```python
from build123d import *

# Parameters (mm, degrees)
SKETCH_1_W          = 200
SKETCH_1_H          = 30
EXTRUDE_1_DEPTH     = 12
SKETCH_2_W          = 12
SKETCH_2_H          = 30
CUT_EXTRUDE_1_DEPTH = 1.5
CUT_EXTRUDE_2_REACH = 103.662
SKETCH_3_R          = 3.5


with BuildPart() as part:
    # 草图1 → 凸台-拉伸1 (new body)
    with BuildSketch(Plane.XY):
        Rectangle(SKETCH_1_W, SKETCH_1_H)
        with BuildLine():
            Line((-92, 11), (-12, 11))
            ThreePointArc((-12, 11), (-9, 8), (-12, 5))
            Line((-12, 5), (-92, 5))
            ThreePointArc((-92, 5), (-95, 8), (-92, 11))
        make_face(mode=Mode.SUBTRACT)
        with BuildLine():
            Line((-92, -11), (-12, -11))
            ThreePointArc((-12, -11), (-9, -8), (-12, -5))
            Line((-12, -5), (-92, -5))
            ThreePointArc((-92, -5), (-95, -8), (-92, -11))
        make_face(mode=Mode.SUBTRACT)
        with BuildLine():
            Line((92, 11), (12, 11))
            ThreePointArc((12, 11), (9, 8), (12, 5))
            Line((12, 5), (92, 5))
            ThreePointArc((92, 5), (95, 8), (92, 11))
        make_face(mode=Mode.SUBTRACT)
        with BuildLine():
            Line((92, -11), (12, -11))
            ThreePointArc((12, -11), (9, -8), (12, -5))
            Line((12, -5), (92, -5))
            ThreePointArc((92, -5), (95, -8), (92, -11))
        make_face(mode=Mode.SUBTRACT)
    extrude(amount=EXTRUDE_1_DEPTH)

    # 草图2 → 切除-拉伸1 (cut)
    with BuildSketch(Plane.XY.offset(12)):
        Rectangle(SKETCH_2_W, SKETCH_2_H)
    extrude(amount=-CUT_EXTRUDE_1_DEPTH, mode=Mode.SUBTRACT)

    # 草图3 → 切除-拉伸2 (cut, up to next)
    with BuildSketch(Plane.XY.offset(10.5), mode=Mode.PRIVATE) as cut_extrude_2_sk1:
        with Locations((0, 9)):
            Circle(SKETCH_3_R)
    cut_extrude_2_tool1 = extrude(cut_extrude_2_sk1.sketch, amount=-CUT_EXTRUDE_2_REACH, mode=Mode.PRIVATE) & part.part
    # 草图3 → 切除-拉伸2 (cut, up to next)
    with BuildSketch(Plane.XY.offset(10.5), mode=Mode.PRIVATE) as cut_extrude_2_sk2:
        with Locations((0, -9)):
            Circle(SKETCH_3_R)
    cut_extrude_2_tool2 = extrude(cut_extrude_2_sk2.sketch, amount=-CUT_EXTRUDE_2_REACH, mode=Mode.PRIVATE) & part.part
    add(cut_extrude_2_tool1.solids().sort_by_distance((0, 9, 10.5))[0], mode=Mode.SUBTRACT)
    add(cut_extrude_2_tool2.solids().sort_by_distance((0, -9, 10.5))[0], mode=Mode.SUBTRACT)


solid = part.part
```
Model file for the job. Use its own axes, mm. A direction names the side the tool comes from. Give positions to 0.01 mm unless a question says otherwise; leave off trailing zeros. Write each loop counter-clockwise with the first axis right and the second up, starting at its lowest first coordinate (ties: lowest second). Pieces come first, ordered by that corner, then holes. Notation, with made-up numbers: (-24.75, -20) - (-18.75, -20) arc R24 ccw to (-18.75, -1) - close; hole circle Ø2 at (54.25, -2.5). An arc over 180 degrees is marked (long way). One line per question, with ' | ' between items. Start each with the question number.
(1) Two-plate mould, pull along Y, no slides. Class faces 4 (the face through (-54, 0, 12)), 5 (the face through (-51, -5, 6)): +Y half, -Y half, draft (parallel to the pull), parting line (faces both ways), or undercut.
(2) 3-axis set-ups, long thin cutter, end or side, ignore diameter. For faces 1 (the face through (-95, -8, 6)), 2 (the face through (-100, 0, 6)), 3 (the face through (0, 0, 10.5)): which of +Z, -Z, +X, -X, +Y, -Y reach the whole face in a straight line?
(3) Pin check, flat tips, straight feed: P1, Ø3, axis at x = -78, y = -8, coming from the +Z side; P2, Ø11, axis at x = 0, y = -9, coming from the +Z side. Stop position of each tip, or through.
(4) Slice it at B-B on x = 0. Write the cut outline in (y, z).
(5) Slice it at C-C on y = -9. Write the cut outline in (x, z).
(6) Slice it at D-D on x = -33. Write the cut outline in (y, z).
(7) Wall check: line 1 along Y through (x, z) = (0, 2.5); line 2 along X through (y, z) = (8, 11.75); line 3 along Y through (x, z) = (44, 11.25). Give the ranges that are in metal, low to high. Write a range as from..to.
(8) Slice it at A-A on z = 7.75. Write the cut outline in (x, y), plus the area to 3 significant figures.
Results below:
1) face 4: draft | face 5: undercut
2) face 1: +Z, -Z | face 2: +Z, -Z, -X, +Y, -Y | face 3: +Z, +Y, -Y
3) P1: through | P2: z = 10.5
4) outline: (-15, 0) - (-12.5, 0) - (-12.5, 10.5) - (-15, 10.5) - close; (-5.5, 0) - (5.5, 0) - (5.5, 10.5) - (-5.5, 10.5) - close; (12.5, 0) - (15, 0) - (15, 10.5) - (12.5, 10.5) - close
5) outline: (-100, 0) - (-94.83, 0) - (-94.83, 12) - (-100, 12) - close; (-9.17, 0) - (-3.5, 0) - (-3.5, 10.5) - (-6, 10.5) - (-6, 12) - (-9.17, 12) - close; (3.5, 0) - (9.17, 0) - (9.17, 12) - (6, 12) - (6, 10.5) - (3.5, 10.5) - close; (94.83, 0) - (100, 0) - (100, 12) - (94.83, 12) - close
6) outline: (-15, 0) - (-11, 0) - (-11, 12) - (-15, 12) - close; (-5, 0) - (5, 0) - (5, 12) - (-5, 12) - close; (11, 0) - (15, 0) - (15, 12) - (11, 12) - close
7) line 1: -15..-12.5, -5.5..5.5, 12.5..15 | line 2: -100..-95, -9..-6, 6..9, 95..100 | line 3: -15..-11, -5..5, 11..15
8) outline: (-100, -15) - (100, -15) - (100, 15) - (-100, 15) - close; hole (-92, -11) - (-12, -11) arc R3 ccw to (-12, -5) - (-92, -5) arc R3 ccw to start; hole (-92, 5) - (-12, 5) arc R3 ccw to (-12, 11) - (-92, 11) arc R3 ccw to start; hole circle Ø7 at (0, -9); hole circle Ø7 at (0, 9); hole (12, -11) - (92, -11) arc R3 ccw to (92, -5) - (12, -5) arc R3 ccw to start; hole (12, 5) - (92, 5) arc R3 ccw to (92, 11) - (12, 11) arc R3 ccw to start | area: 3,890 mm^2
